Could you check a few things on this drawing? It's one solid part, dimensions in mm from its lowest x, y, z. A direction names the side the tool comes from. Give positions to 0.01 mm unless a question says otherwise; leave off trailing zeros. Loops run counter-clockwise (first coordinate to the right, second up) from the corner with the lowest first, then second, coordinate; pieces in that order, holes last. Notation, with made-up numbers: (4, 71) - (53, 71) arc R19 ccw to (53, 84) - close; hole circle Ø6 at (26, 70). An arc over 180 degrees is marked (long way). Use CSV: the item, a comma, the result in double quotes.
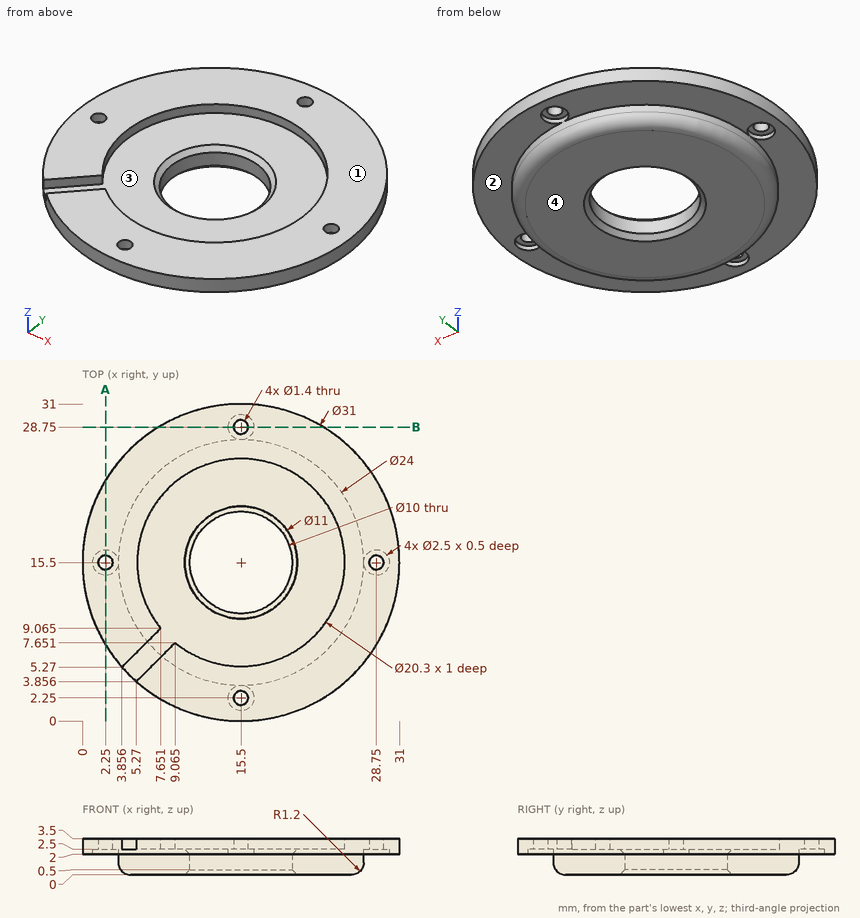
1) Suppose I cut it at A-A (x = 2.25). Please give me the cut outline in (y, z).
Answer below:
outline,"(7.46, 2) - (14.25, 2) - (14.25, 2.5) - (14.8, 2.5) - (14.8, 3.5) - (7.46, 3.5) - close; (16.2, 2.5) - (16.75, 2.5) - (16.75, 2) - (23.54, 2) - (23.54, 3.5) - (16.2, 3.5) - close"
2) I need wall thicknesses on line 1 along Y through (x, z) = (15.5, 3.05); line 2 along Y through (x, z) = (16, 3.3) (1 decimal). Which ranges of each line are inside material? Lowest first, please.
Answer below:
line 1,"y = 0 to 1.55, 2.95 to 5.35, 25.65 to 28.05, 29.45 to 31"
line 2,"y = 0 to 1.8, 2.7 to 5.4, 25.6 to 28.3, 29.2 to 31"
3) We'd pull the mould along X, two halves only. Please class the marked faces 3 and 4: +X half, -X half, draft (parallel to the pull), parting line (faces both ways), or undercut.
Answer below:
face 3,"undercut"
face 4,"draft"
4) I'm going to push flat-ended pins straight in: P1, Ø3, axis at x = 3, y = 15.5, coming from the -Z side; P2, Ø2, axis at x = 15.5, y = 28.75, coming from the -Z side; P3, Ø0.8, axis at x = 15.5, y = 2.25, coming from the -Z side; P4, Ø3, axis at x = 2.25, y = 15.5, coming from the -Z side (1 decimal). Where does each tip first touch, or does it pass through?
Answer below:
P1,"stops at z = 0.02"
P2,"stops at z = 2.5"
P3,"passes through"
P4,"stops at z = 0.5"
5) Which directions (+Z, -Z, +X, -X, +Y, -Y) give clear straight access to the entire face, cutting with the end or side of a thin tool? Please do the marked faces 1 and 2.
Answer below:
face 1,"+Z, +X, -X, +Y, -Y"
face 2,"-Z"
